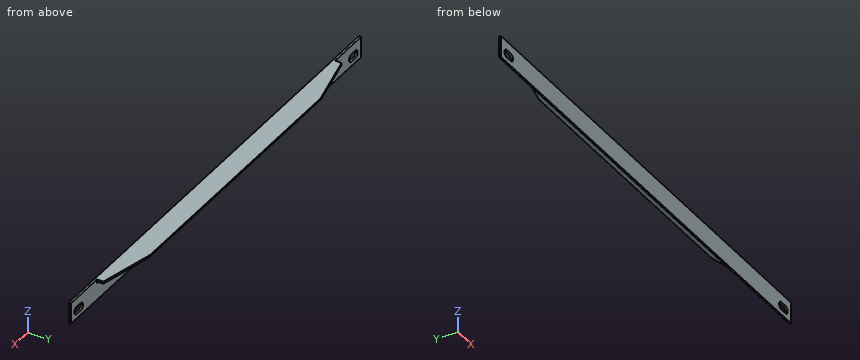
```python
from build123d import *

# Parameters (mm, degrees)
HOT_ROLLED_EQUAL_LEG_ANGLE_STEEL_GB_T97_DEPTH = 1113
CUT_EXTRUDE1_REACH                            = 562.551
CUT_EXTRUDE2_REACH                            = 562.551
SKETCH16_W                                    = 100
SKETCH16_H                                    = 10.5
CUT_EXTRUDE3_DEPTH                            = 561.550845151
CUT_EXTRUDE3_DEPTH_BACK                       = 561.550845151


with BuildPart() as part:
    # Sketch11 → Hot-rolled equal-leg angle steel (gb t9787-1988) 50×5(1) (new body)
    with BuildSketch(Plane.YZ.offset(-556.5)):
        with BuildLine():
            Line((50, 0), (0, 0))
            Line((0, 0), (0, -50))
            Line((0, -50), (3.333333333, -50))
            ThreePointArc((3.333333333, -50), (4.511844635, -49.511844635), (5, -48.333333333))
            Line((5, -48.333333333), (5, -10.5))
            ThreePointArc((5, -10.5), (6.610912703, -6.610912703), (10.5, -5))
            Line((10.5, -5), (48.333333333, -5))
            ThreePointArc((48.333333333, -5), (49.511844635, -4.511844635), (50, -3.333333333))
            Line((50, -3.333333333), (50, 0))
        make_face()
    extrude(amount=HOT_ROLLED_EQUAL_LEG_ANGLE_STEEL_GB_T97_DEPTH)

    # Sketch13 → Cut-Extrude1 (cut, up to next)
    with BuildSketch(Plane(origin=(0, 5, 0), x_dir=(1, 0, 0), z_dir=(0, 1, 0)), mode=Mode.PRIVATE) as cut_extrude1_sk1:
        with BuildLine():
            Line((-534, 38.416666667), (-519, 38.416666667))
            ThreePointArc((-519, 38.416666667), (-510, 29.416666667), (-519, 20.416666667))
            Line((-519, 20.416666667), (-534, 20.416666667))
            ThreePointArc((-534, 20.416666667), (-543, 29.416666667), (-534, 38.416666667))
        make_face()
    cut_extrude1_tool1 = extrude(cut_extrude1_sk1.sketch, amount=-CUT_EXTRUDE1_REACH, mode=Mode.PRIVATE) & part.part
    # Sketch13 → Cut-Extrude1 (cut, up to next)
    with BuildSketch(Plane(origin=(0, 5, 0), x_dir=(1, 0, 0), z_dir=(0, 1, 0)), mode=Mode.PRIVATE) as cut_extrude1_sk2:
        with BuildLine():
            Line((534, 20.416666667), (519, 20.416666667))
            ThreePointArc((519, 20.416666667), (510, 29.416666667), (519, 38.416666667))
            Line((519, 38.416666667), (534, 38.416666667))
            ThreePointArc((534, 38.416666667), (543, 29.416666667), (534, 20.416666667))
        make_face()
    cut_extrude1_tool2 = extrude(cut_extrude1_sk2.sketch, amount=-CUT_EXTRUDE1_REACH, mode=Mode.PRIVATE) & part.part
    add(cut_extrude1_tool1.solids().sort_by_distance((-526.5, 5, -29.416667))[0], mode=Mode.SUBTRACT)
    add(cut_extrude1_tool2.solids().sort_by_distance((526.5, 5, -29.416667))[0], mode=Mode.SUBTRACT)

    # Sketch16 → Cut-Extrude2 (cut, up to next)
    with BuildSketch(Plane(origin=(0, 5, 0), x_dir=(1, 0, 0), z_dir=(0, 1, 0)), mode=Mode.PRIVATE) as cut_extrude2_sk1:
        with Locations((506.5, 5.25)):
            Rectangle(SKETCH16_W, SKETCH16_H)
    cut_extrude2_tool1 = extrude(cut_extrude2_sk1.sketch, amount=CUT_EXTRUDE2_REACH, mode=Mode.PRIVATE) & part.part
    # Sketch16 → Cut-Extrude2 (cut, up to next)
    with BuildSketch(Plane(origin=(0, 5, 0), x_dir=(1, 0, 0), z_dir=(0, 1, 0)), mode=Mode.PRIVATE) as cut_extrude2_sk2:
        with Locations((-506.5, 5.25)):
            Rectangle(SKETCH16_W, SKETCH16_H)
    cut_extrude2_tool2 = extrude(cut_extrude2_sk2.sketch, amount=CUT_EXTRUDE2_REACH, mode=Mode.PRIVATE) & part.part
    add(cut_extrude2_tool1.solids().sort_by_distance((506.5, 5, -5.25))[0], mode=Mode.SUBTRACT)
    add(cut_extrude2_tool2.solids().sort_by_distance((-506.5, 5, -5.25))[0], mode=Mode.SUBTRACT)

    # Sketch17 → Cut-Extrude3 (cut, two sides: drawn at the far end of the back side and taken through both)
    with BuildSketch(Plane(origin=(0, 0, -5), x_dir=(-1, 0, 0), z_dir=(0, 0, -1)).offset(-CUT_EXTRUDE3_DEPTH_BACK)):
        Polygon((326.5, 50), (456.5, 50), (456.5, 20), align=None)
        Polygon((-456.5, 20), (-326.5, 50), (-456.5, 50), align=None)
    extrude(amount=CUT_EXTRUDE3_DEPTH + CUT_EXTRUDE3_DEPTH_BACK, mode=Mode.SUBTRACT)


solid = part.part
```
Could you check a few things on this model? Use its own coordinates, in mm. Round coordinates to 2 decimals unless told otherwise and drop trailing zeros. Write each loop counter-clockwise with the first axis right and the second up, starting at its lowest first coordinate (ties: lowest second). Pieces come first, ordered by that corner, then holes.
(1) For pin 1 (19 mm diameter, centred on x = -72.5, y = 37, fed in from -Z); pin 2 (3 mm diameter, centred on y = 14.5, z = -4.5, fed in from +X); pin 3 (1 mm diameter, centred on y = 6.5, z = -37, fed in from +X); pin 4 (24 mm diameter, centred on x = -93.5, z = -23.5, fed in from +Y), each with a flat end and sliding along its axis, tell me the tip position at first contact or that it passes through.
Findings below:
pin 1: stops at z = -5
pin 2: stops at x = 456.5
pin 3: passes through
pin 4: stops at y = 5
(2) If I drill on probe 1 along Y at (x, z) = (478, -26); probe 2 along Z at (x, y) = (402, 27); probe 3 along X at (y, z) = (5.5, -5), over which ranges is the centre line in solid material (lowest first)?
Findings below:
probe 1: y = 0 to 5
probe 2: z = -5 to 0
probe 3: x = -456.5 to 456.5
(3) Suppose I cut it at A-A on x = 118. Write out the boundary of the cut face in (y, z), and give its area (3 significant figures).
Findings below:
outline: (0, -50) - (3.33, -50) arc R1.67 ccw to (5, -48.33) - (5, -10.5) arc R5.5 cw to (10.5, -5) - (48.33, -5) arc R1.67 ccw to (50, -3.33) - (50, 0) - (0, 0) - close
area: 480 mm2
(4) Suppose I cut it at B-B on y = 38. Write out the boundary of the cut face in (x, z), and give its area (4 significant figures).
Findings below:
outline: (-378.5, -5) - (378.5, -5) - (378.5, 0) - (-378.5, 0) - close
area: 3,785 mm2
